Part model, mm, in its own coordinate system. A direction names the side the tool comes from. Coordinates: 2 decimals unless noted, no trailing zeros. Write each loop counter-clockwise with the first axis right and the second up, starting at its lowest first coordinate (ties: lowest second). Pieces come first, ordered by that corner, then holes. Notation, with made-up numbers: M -38.75,77.25 L -31.75,77.25 A15 ccw -31.75,93.25 Z; hole C 81,-25.5 d10. An arc over 180 degrees is marked long. Use a Markdown table: item, result. Add a question column.
Q1. Slice it at D-D on y = 8.75. Write the cut outline in (x, z).
Q2. Slice it at B-B on z = 0.5. Write the cut outline in (x, y).
Q3. Wall check: L1, parallel to X at y = 0.95, z = 2.5; L2, parallel to X at y = 1.3, z = 2.5; L3, parallel to Y at x = 11, z = 3.45. Give the ranges that are in metal, low to high. Write a range as from..to.
Q4. Pin check, flat tips, straight feed: pin 1 Ø3 at (x, y) = (3.5, 4) entering from -Z; pin 2 Ø2 at (y, z) = (5, 4) entering from -X; pin 3 Ø1.8 at (x, z) = (13.33, 2.5) entering from -Y; pin 4 Ø3 at (y, z) = (5, 3) entering from -X. Stop position of each tip, or through.
Q5. Slice it at C-C on x = 10.5. Write the cut outline in (y, z).
Q6. Tool access for faces 4 (the flat face through (12, 2, 2)), 5 (the cylindrical face through (-2, 6, 3)): list every direction of +Z, -Z, +X, -X, +Y, -Y with a clear straight run to the whole face (end or side of a thin tool).
Q7. Slice it at A-A on z = 2.5. Write the cut outline in (x, y).
Q8. Mould opens along X. For faces 1 (the flat face through (17.083, 1, 2)), 2 (the flat face through (-16, 2, 2)), 3 (the cylindrical face through (12.357, 1.014, 2.283)) say: released by +X, released by -X, zero draft, split by the parting line, or undercut.
from build123d import *

# Parameters (mm, degrees)
BOSS_EXTRUDE1_DEPTH = 5
SKETCH3_R           = 1
CUT_EXTRUDE2_DEPTH  = 7
SKETCH4_R           = 6
CUT_EXTRUDE3_DEPTH  = 25.38777855


with BuildPart() as part:
    # Sketch2 → Boss-Extrude1 (new body)
    with BuildSketch(Plane.XY):
        with BuildLine():
            Line((9.583170828, 0), (17.083170828, 0))
            Line((17.083170828, 0), (17.083170828, 2))
            Line((17.083170828, 2), (9.407922481, 2))
            ThreePointArc((9.407922481, 2), (-1.916829172, 11.5), (-13.241580825, 2))
            Line((-13.241580825, 2), (-20.916829172, 2))
            Line((-20.916829172, 2), (-20.916829172, 0))
            Line((-20.916829172, 0), (-13.416829172, 0))
            Line((-13.416829172, 0), (-7.916829172, 0))
            Line((-7.916829172, 0), (4.083170828, 0))
            Line((4.083170828, 0), (9.583170828, 0))
        make_face()
    extrude(amount=BOSS_EXTRUDE1_DEPTH)

    # Sketch3 → Cut-Extrude2 (cut)
    with BuildSketch(Plane(origin=(0, 2, 0), x_dir=(1, 0, 0), z_dir=(0, 1, 0))):
        with Locations(Location((-17.166829172, -2.5, 0), (0, 0, 270))):
            Circle(SKETCH3_R)
        with Locations(Location((13.333170828, -2.5, 0), (0, 0, 270))):
            Circle(SKETCH3_R)
    extrude(amount=-CUT_EXTRUDE2_DEPTH, mode=Mode.SUBTRACT)

    # Sketch4 → Cut-Extrude3 (cut, through all)
    with BuildSketch(Plane.XY.offset(5)):
        with Locations((-1.916829172, 0)):
            Circle(SKETCH4_R)
    extrude(amount=-CUT_EXTRUDE3_DEPTH, mode=Mode.SUBTRACT)


solid = part.part
Recorded:
| question | item | result |
|---|---|---|
| 1 | outline | M -9.38,0 L 5.55,0 L 5.55,5 L -9.38,5 Z |
| 2 | outline | M -20.92,0 L -7.92,0 A6 cw 4.08,0 L 17.08,0 L 17.08,2 L 9.41,2 A11.5 ccw -13.24,2 L -20.92,2 Z |
| 3 | L1 | -20.92..-18.17, -16.17..-7.84, 4.01..12.33, 14.33..17.08 |
| 3 | L2 | -20.92..-18.17, -16.17..-7.77, 3.94..12.33, 14.33..17.08 |
| 3 | L3 | 0..2 |
| 4 | pin 1 | z = 0 |
| 4 | pin 2 | x = -12.7 |
| 4 | pin 3 | through |
| 4 | pin 4 | x = -12.87 |
| 5 | outline | M 0,0 L 2,0 L 2,5 L 0,5 Z |
| 6 | face 4 | +Z, -Z, +X, +Y |
| 6 | face 5 | +Z, -Z, -Y |
| 7 | outline | M -20.92,0 L -18.17,0 L -18.17,2 L -20.92,2 Z; M -16.17,0 L -7.92,0 A6 cw 4.08,0 L 12.33,0 L 12.33,2 L 9.41,2 A11.5 ccw -13.24,2 L -16.17,2 Z; M 14.33,0 L 17.08,0 L 17.08,2 L 14.33,2 Z |
| 8 | face 1 | released by +X |
| 8 | face 2 | zero draft |
| 8 | face 3 | undercut |
